```python
from build123d import *

# Parameters (mm, degrees)
SKETCH1_R           = 5
BOSS_EXTRUDE1_DEPTH = 40
CUT_EXTRUDE1_DEPTH  = 3


with BuildPart() as part:
    # Sketch1 → Boss-Extrude1 (new body)
    with BuildSketch(Plane.XY):
        Circle(SKETCH1_R)
    extrude(amount=BOSS_EXTRUDE1_DEPTH)

    # Sketch2 → Cut-Extrude1 (cut)
    with BuildSketch(Plane(origin=(0, 5, 0), x_dir=(1, 0, 0), z_dir=(0, 1, 0))):
        with BuildLine():
            Line((-1.876815102, -12), (-1.876815102, -2.691594063))
            ThreePointArc((-1.876815102, -2.691594063), (0, -0.814778961), (1.876815102, -2.691594063))
            Line((1.876815102, -2.691594063), (1.876815102, -12))
            ThreePointArc((1.876815102, -12), (0, -13.876815102), (-1.876815102, -12))
        make_face()
    extrude(amount=-CUT_EXTRUDE1_DEPTH, mode=Mode.SUBTRACT)


solid = part.part
```
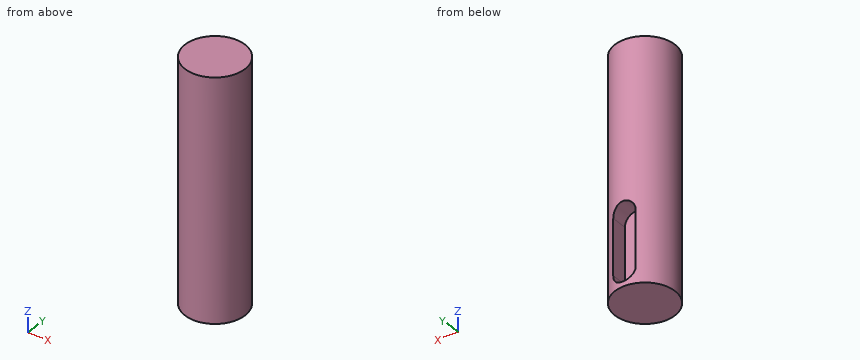
For this review, take the finished solid that the model builds, in its own axes (mm). Give positions to 0.01 mm unless a question says otherwise; leave off trailing zeros. Write each loop counter-clockwise with the first axis right and the second up, starting at its lowest first coordinate (ties: lowest second). Pieces come first, ordered by that corner, then holes.
Item 1: Take a section at B-B (x = 0). Give the boundary of the cut face in (y, z).
Item 2: Take a section at D-D (y = -4). Give the boundary of the cut face in (x, z).
Item 3: Insertion check: P1, Ø4, axis at x = 0, z = 10, coming from the +Y side; P2, Ø2, axis at y = 3, z = 5.5, coming from the +X side; P3, Ø1.3, axis at y = 4, z = 9, coming from the -X side. Each pin has a flat end and moves straight along its axis. Give the tip position at first contact, or say it passes through.
Item 4: Wall thickness on probe 1 along Z at (x, y) = (-1.25, 2.5); probe 2 along Z at (x, y) = (1.5, 2.75); probe 3 along Y at (x, z) = (3, 34): over which ranges is each line inside the solid? List them lowest first.
Item 5: Take a section at A-A (y = 3). Give the boundary of the cut face in (x, z), and give its area (3 significant figures).
Item 6: Take a section at C-C (z = 33.5). Give the boundary of the cut face in (x, y).
Established:
1. outline: (-5, 0) - (5, 0) - (5, 0.81) - (2, 0.81) - (2, 13.88) - (5, 13.88) - (5, 40) - (-5, 40) - close
2. outline: (-3, 0) - (3, 0) - (3, 40) - (-3, 40) - close
3. P1: stops at y = 4.63
3. P2: stops at x = 4.58
3. P3: stops at x = -3.71
4. probe 1: z = 0 to 1.29, 13.4 to 40
4. probe 2: z = 0 to 1.56, 13.13 to 40
4. probe 3: y = -4 to 4
5. outline: (-4, 0) - (4, 0) - (4, 40) - (-4, 40) - close; hole (-1.88, 2.69) arc R1.88 ccw to (1.88, 2.69) - (1.88, 12) arc R1.88 ccw to (-1.88, 12) - close
5. area: 274 mm2
6. outline: circle Ø10 at (0, 0)
